from build123d import *

# Parameters (mm, degrees)
BOSS_EXTRUDE1_DEPTH = 500
CUT_EXTRUDE1_REACH  = 504.888
SKETCH_1_R          = 6.5


with BuildPart() as part:
    # Sketch1 → Boss-Extrude1 (new body)
    with BuildSketch(Plane.XY):
        with BuildLine():
            Line((0, 0), (0, 40))
            Line((0, 40), (2.666666667, 40))
            ThreePointArc((2.666666667, 40), (3.609475708, 39.609475708), (4, 38.666666667))
            Line((4, 38.666666667), (4, 9))
            ThreePointArc((4, 9), (5.464466094, 5.464466094), (9, 4))
            Line((9, 4), (38.666666667, 4))
            ThreePointArc((38.666666667, 4), (39.609475708, 3.609475708), (40, 2.666666667))
            Line((40, 2.666666667), (40, 0))
            Line((40, 0), (0, 0))
        make_face()
    extrude(amount=BOSS_EXTRUDE1_DEPTH)

    # 草图1 → Cut-Extrude1 (cut, up to next)
    with BuildSketch(Plane(origin=(0, 4, 0), x_dir=(1, 0, 0), z_dir=(0, 1, 0)), mode=Mode.PRIVATE) as cut_extrude1_sk1:
        with Locations(Location((25, -75, 0), (0, 0, 180))):
            Circle(SKETCH_1_R)
    cut_extrude1_tool1 = extrude(cut_extrude1_sk1.sketch, amount=-CUT_EXTRUDE1_REACH, mode=Mode.PRIVATE) & part.part
    add(cut_extrude1_tool1.solids().sort_by_distance((25, 4, 75))[0], mode=Mode.SUBTRACT)


solid = part.part
For this review, take the finished solid that the model builds, in its own axes (mm). A direction names the side the tool comes from. Coordinates: 2 decimals unless noted, no trailing zeros. Loops run counter-clockwise (first coordinate to the right, second up) from the corner with the lowest first, then second, coordinate; pieces in that order, holes last. Notation, with made-up numbers: (-35.5, 51) - (-30.5, 51) arc R7 ccw to (-30.5, 62) - close; hole circle Ø11 at (59, 80.5). An arc over 180 degrees is marked (long way). Use a Markdown table: item, result. Add a question column.
Item 1: We need section C-C (z = 75). Give the boundary of the cut face in (x, y).
Item 2: Mouldability with a two-part tool opening along Z and no side actions: class faces 3 (the face through (12.7, 3.8, 500)), 4 (the face through (26.409, 2.028, 68.655)), 5 (the face through (12.7, 3.8, 0)), 6 (the face through (20, 0, 246)) as pulls with the +Z half, pulls with the -Z half, needs draft (parallel to the pull), parting line crosses it, or undercut.
Item 3: For line 1 (Z direction, x = 25, y = 2.4); line 2 (Y direction, x = 38.5, z = 257.5), list the stretches that pass through material, from the lowest coordinate up.
Item 4: Insertion check: pin 1 Ø3 at (y, z) = (4.5, 324) entering from +X; pin 2 Ø2 at (y, z) = (33.5, 108) entering from +X; pin 3 Ø8 at (x, y) = (11.5, 23.5) entering from -Z; pin 4 Ø9 at (x, z) = (22, 182) entering from +Y. Each pin has a flat end and moves straight along its axis. Give the tip position at first contact, or say it passes through.
Item 5: Tool access review of faces 1 (the face through (4, 24, 246)), 2 (the face through (0, 20, 246)): name each direction out of +Z, -Z, +X, -X, +Y, -Y from which nothing blocks a thin tool from reaching the whole face with its end or side.
Item 6: We need section D-D (y = 22.5). Give the boundary of the cut face in (x, z), and give its area (3 significant figures).
Item 7: We need section B-B (z = 247.5). Give the boundary of the cut face in (x, y).
Item 8: We need section A-A (x = 25). Give the boundary of the cut face in (y, z), and give its area (3 significant figures).
Results list:
| question | item | result |
|---|---|---|
| 1 | outline | (0, 0) - (18.5, 0) - (18.5, 4) - (9, 4) arc R5 cw to (4, 9) - (4, 38.67) arc R1.33 ccw to (2.67, 40) - (0, 40) - close; (31.5, 0) - (40, 0) - (40, 2.67) arc R1.33 ccw to (38.67, 4) - (31.5, 4) - close |
| 2 | face 3 | pulls with the +Z half |
| 2 | face 4 | undercut |
| 2 | face 5 | pulls with the -Z half |
| 2 | face 6 | needs draft |
| 3 | line 1 | z = 0 to 68.5, 81.5 to 500 |
| 3 | line 2 | y = 0 to 4 |
| 4 | pin 1 | stops at x = 39.96 |
| 4 | pin 2 | stops at x = 4 |
| 4 | pin 3 | passes through |
| 4 | pin 4 | stops at y = 4 |
| 5 | face 1 | +Z, -Z, +X, +Y |
| 5 | face 2 | +Z, -Z, -X, +Y, -Y |
| 6 | outline | (0, 0) - (4, 0) - (4, 500) - (0, 500) - close |
| 6 | area | 2,000 mm^2 |
| 7 | outline | (0, 0) - (40, 0) - (40, 2.67) arc R1.33 ccw to (38.67, 4) - (9, 4) arc R5 cw to (4, 9) - (4, 38.67) arc R1.33 ccw to (2.67, 40) - (0, 40) - close |
| 8 | outline | (0, 0) - (4, 0) - (4, 68.5) - (0, 68.5) - close; (0, 81.5) - (4, 81.5) - (4, 500) - (0, 500) - close |
| 8 | area | 1,950 mm^2 |
